Could you check a few things on this model? Use its own coordinates, in mm. A direction names the side the tool comes from. Coordinates: 2 decimals unless noted, no trailing zeros. Loops run counter-clockwise (first coordinate to the right, second up) from the corner with the lowest first, then second, coordinate; pieces in that order, holes last.
from build123d import *

# Parameters (mm, degrees)
SKETCH1_W     = 20
SKETCH1_H     = 30
SKETCH1_W_2   = 17.5
SKETCH1_H_2   = 3
CHAMFER1_SIZE = 2
CHAMFER2_SIZE = 2


with BuildPart() as part:
    # Sketch1 → Revolve1 (revolve)
    with BuildSketch(Plane.XY, mode=Mode.PRIVATE) as revolve1_sk:
        Polygon((0, -35.605263158), (0, -5.605263158), (-17.5, -5.605263158), (-25, -5.605263158), (-25, -35.605263158), align=None)
        with Locations((-10, 12.394736842)):
            Rectangle(SKETCH1_W, SKETCH1_H)
        with Locations((-8.75, -4.105263158)):
            Rectangle(SKETCH1_W_2, SKETCH1_H_2)
    revolve(revolve1_sk.sketch.rotate(Axis((0, 37.5, 0), (0, -1, 0)), 270), axis=Axis((0, 37.5, 0), (0, -1, 0)))

    # Chamfer1
    chamfer1_edges = [part.edges().sort_by_distance(p)[0] for p in [
        (0, 27.394736842, -20),
    ]]
    chamfer(chamfer1_edges, length=CHAMFER1_SIZE)

    # Chamfer2
    chamfer2_edges = [part.edges().sort_by_distance(p)[0] for p in [
        (0, -35.605263158, -25),
    ]]
    chamfer(chamfer2_edges, length=CHAMFER2_SIZE)


solid = part.part
(1) I need wall thicknesses on probe 1 along Z at (x, y) = (15, -31); probe 2 along Y at (x, z) = (21, -6); probe 3 along X at (y, z) = (-12.5, 15.5). Which ranges of each line are inside material? Lowest first, please.
Answers:
probe 1: z = -20 to 20
probe 2: y = -35.61 to -5.61
probe 3: x = -19.62 to 19.62
(2) Imagine slicing it at B-B, the plane x = 0. Write out the boundary of the cut face in (y, z).
Answers:
outline: (-35.61, -23) - (-33.61, -25) - (-5.61, -25) - (-5.61, -17.5) - (-2.61, -17.5) - (-2.61, -20) - (25.39, -20) - (27.39, -18) - (27.39, 18) - (25.39, 20) - (-2.61, 20) - (-2.61, 17.5) - (-5.61, 17.5) - (-5.61, 25) - (-33.61, 25) - (-35.61, 23) - close
(3) Imagine slicing it at D-D, the plane y = 21. Write out the boundary of the cut face in (x, z), and give its area (3 significant figures).
Answers:
outline: circle Ø40 at (0, 0)
area: 1,260 mm2
(4) Imagine slicing it at A-A, the plane z = 0. Write out the boundary of the cut face in (x, y).
Answers:
outline: (-25, -33.61) - (-23, -35.61) - (23, -35.61) - (25, -33.61) - (25, -5.61) - (17.5, -5.61) - (17.5, -2.61) - (20, -2.61) - (20, 25.39) - (18, 27.39) - (-18, 27.39) - (-20, 25.39) - (-20, -2.61) - (-17.5, -2.61) - (-17.5, -5.61) - (-25, -5.61) - close
(5) For pin 1 (4 mm diameter, centred on y = 8.5, z = -5, fed in from +X); pin 2 (12 mm diameter, centred on x = -13, y = -3.5, fed in from +Z); pin 3 (5 mm diameter, centred on y = 2.5, z = -10, fed in from -X), each with a flat end and sliding along its axis, tell me the tip position at first contact or that it passes through.
Answers:
pin 1: stops at x = 19.77
pin 2: stops at z = 23.89
pin 3: stops at x = -18.54
(6) Which directions (+Z, -Z, +X, -X, +Y, -Y) give clear straight access to the entire face, cutting with the end or side of a thin tool? Please do faces 4 (the face through (19.524, 11.591, -4.336)), 5 (the face through (0, 27.395, 0)), 6 (the face through (10.648, -4.084, -13.887)).
Answers:
face 4: +Y
face 5: +Z, -Z, +X, -X, +Y
face 6: none
(7) Imagine slicing it at C-C, the plane y = -3.5. Write out the boundary of the cut face in (x, z).
Answers:
outline: circle Ø35 at (0, 0)
(8) We'd pull the mould along Y, two halves only. Please class faces 1 (the face through (-5.44, 27.27, 17.29)), 2 (the face through (18, -2.605, 0)), 3 (the face through (-7.509, -19.801, 23.846)): +Y half, -Y half, draft (parallel to the pull), parting line (faces both ways), or undercut.
Answers:
face 1: +Y half
face 2: undercut
face 3: draft
